Part model, mm, in its own coordinate system. A direction names the side the tool comes from. Round coordinates to 2 decimals unless told otherwise and drop trailing zeros. Write each loop counter-clockwise with the first axis right and the second up, starting at its lowest first coordinate (ties: lowest second). Pieces come first, ordered by that corner, then holes. Notation, with made-up numbers: M 67,9.5 L 101,9.5 A14 cw 101,36.5 Z; hole C 54.5,42.5 d9. An arc over 180 degrees is marked long. Use one line per item in the form item = value. Start each with the question number.
Item 1: Mould opens along X. For faces 1 (the face through (136.4, 43.2, 0.7)), 2 (the face through (111, 85, 1.5)), 3 (the face through (38.953, 73.037, 0.74)) say: +X half, -X half, draft (parallel to the pull), parting line (faces both ways), or undercut.
Item 2: Which spindle directions (+Z, -Z, +X, -X, +Y, -Y) get a long thin tool onto all of the face, cutting with end or side? Do faces 4 (the face through (267.15, 86.99, 0.74)), 5 (the face through (111, 85, 0)). Say none if no direction does.
Item 3: Cut at B-B, the plane y = 120. Give the cut face in (x, z), then the cut area to 3 significant figures.
Item 4: Cut at A-A, the plane z = 0.4. Give the cut face in (x, y).
Item 5: Flat gauge pin, fed straight in: pin 1 Ø0.8 at (y, z) = (-23, 0.5) entering from -X. Where does the tip first touch, or does it go through?
Item 6: Cut at C-C, the plane x = 251. Give the cut face in (y, z), then the cut area to 3 significant figures.
Item 7: Probe L1, parallel to X at y = -19.5, z = 0.15; L2, parallel to Y at x = 180, z = 1.25; L3, parallel to X at y = 51.5, z = 0.7. List the from-to ranges inside material, lowest first.
from build123d import *

# Parameters (mm, degrees)
BOSS_EXTRUDE1_DEPTH = 1.5


with BuildPart() as part:
    # Sketch1 → Boss-Extrude1 (new body)
    with BuildSketch(Plane.XY):
        with BuildLine():
            Line((0, 0), (79.011764706, 148.147058824))
            ThreePointArc((79.011764706, 148.147058824), (80.299264856, 149.50122524), (82.1, 150))
            Line((82.1, 150), (276.5, 150))
            ThreePointArc((276.5, 150), (278.974873734, 148.974873734), (280, 146.5))
            Line((280, 146.5), (280, -90))
            Line((280, -90), (270, -90))
            Line((270, -90), (270, 80))
            ThreePointArc((270, 80), (267.071067812, 87.071067812), (260, 90))
            Line((260, 90), (170.608346172, 90))
            ThreePointArc((170.608346172, 90), (165.716771832, 88.721955083), (162.075527836, 85.214500095))
            Line((162.075527836, 85.214500095), (110, 0))
            Line((110, 0), (0, 0))
        make_face()
    extrude(amount=BOSS_EXTRUDE1_DEPTH)


solid = part.part
Model answer:
q1.face_1 = undercut
q1.face_2 = draft
q1.face_3 = -X half
q2.face_4 = +Z, -Z, -Y
q2.face_5 = -Z, +X, -X, +Y, -Y
q3.outline = M 64,0 L 280,0 L 280,1.5 L 64,1.5 Z
q3.area = 324 mm²
q4.outline = M 0,0 L 110,0 L 162.08,85.21 A10 cw 170.61,90 L 260,90 A10 cw 270,80 L 270,-90 L 280,-90 L 280,146.5 A3.5 ccw 276.5,150 L 82.1,150 A3.5 ccw 79.01,148.15 Z
q5.pin_1 = 270
q6.outline = M 90,0 L 150,0 L 150,1.5 L 90,1.5 Z
q6.area = 90.0 mm²
q7.L1 = 270 to 280
q7.L2 = 90 to 150
q7.L3 = 27.47 to 141.47, 270 to 280
